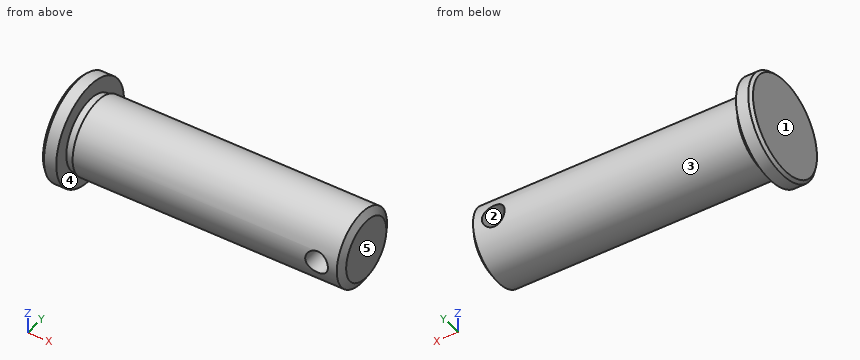
from build123d import *

# Parameters (mm, degrees)
CHAMFER_1_SIZE           = 1.5
CHAMFER_2_SIZE           = 4
CHAMFER_2_SIZE2          = 2.309401077
CUT_EXTRUDE_1_DEPTH      = 159.663165227
CUT_EXTRUDE_1_DEPTH_BACK = 159.663165227
SKETCH_2_R               = 6


with BuildPart() as part:
    # 草图1 → 旋转1 (revolve)
    with BuildSketch(Plane.XY, mode=Mode.PRIVATE) as revolve_1_sk:
        Polygon((0, 0), (154, 0), (154, 20), (12, 20), (12, 19), (8, 19), (8, 27), (0, 27), align=None)
    revolve(revolve_1_sk.sketch.rotate(Axis((-105.652173913, 0, 0), (1, 0, 0)), 90), axis=Axis((-105.652173913, 0, 0), (1, 0, 0)))

    # 倒角1
    chamfer_1_edges = [part.edges().sort_by_distance(p)[0] for p in [
        (0, 0, -27),
    ]]
    chamfer(chamfer_1_edges, length=CHAMFER_1_SIZE)

    # 倒角2
    chamfer_2_edges = [part.edges().sort_by_distance(p)[0] for p in [
        (154, 0, -20),
    ]]
    chamfer_2_side = [part.faces().sort_by_distance(p)[0] for p in [
        (154, 0, 0),
    ]]
    chamfer(chamfer_2_edges, length=CHAMFER_2_SIZE, length2=CHAMFER_2_SIZE2, reference=chamfer_2_side[0])

    # 草图2 → 切除-拉伸1 (cut, two sides: drawn at the far end of the back side and taken through both)
    with BuildSketch(Plane(origin=(0, 0, 0), x_dir=(1, 0, 0), z_dir=(0, 1, 0)).offset(-CUT_EXTRUDE_1_DEPTH_BACK)):
        with Locations(Location((141, 0, 0), (0, 0, 270))):
            Circle(SKETCH_2_R)
    extrude(amount=CUT_EXTRUDE_1_DEPTH + CUT_EXTRUDE_1_DEPTH_BACK, mode=Mode.SUBTRACT)


solid = part.part
Input: part model. Units: mm. Frame: model coordinates. Face numbers are marked on the shaded views. A direction names the side the tool comes from. Round coordinates to 2 decimals unless told otherwise and drop trailing zeros. Write each loop counter-clockwise with the first axis right and the second up, starting at its lowest first coordinate (ties: lowest second). Pieces come first, ordered by that corner, then holes.
1) Draft query along Z for the marked faces 1, 2 and 3. Return one class per face: pulls with the +Z half, pulls with the -Z half, needs draft (parallel to the pull), parting line crosses it, or undercut.
2) Reachability of the marked faces 4 and 5 from +Z, -Z, +X, -X, +Y, -Y: full face, straight path, thin tool, end or side. Return the list, or none.
3) Cut plane D-D (x = 141). Return the cut outline in (y, z).
4) Cut plane C-C (x = 36.5). Return the cut outline in (y, z), then the cut area to 3 significant figures.
5) Cut plane B-B (y = 0). Return the cut outline in (x, z), then the cut area to 3 significant figures.
6) Ray query, L1, parallel to X at y = -4, z = 0; L2, parallel to X at y = 6, z = -22; L3, parallel to Z at x = 141, y = -8. Return the intervals inside material, ascending.
7) Cut plane A-A (z = 0). Return the cut outline in (x, y).
8) Contact query for flat-ended pins moving along their axis: P1, Ø5, axis at x = 110, z = -4.5, coming from the -Y side; P2, Ø2, axis at x = 38.5, y = 2.5, coming from the -Z side; P3, Ø1.5, axis at x = 138, z = 7, coming from the +Y side. Output: stop coordinate, or through.
Geometry says:
1. face 1: needs draft
1. face 2: undercut
1. face 3: parting line crosses it
2. face 4: none
2. face 5: +Z, -Z, +X, +Y, -Y
3. outline: (-19.08, -6) arc R20 ccw to (19.08, -6) - close; (-19.08, 6) - (19.08, 6) arc R20 ccw to start
4. outline: circle Ø40 at (0, 0)
4. area: 1,260 mm2
5. outline: (0, -25.5) - (1.5, -27) - (8, -27) - (8, -19) - (12, -19) - (12, -20) - (151.69, -20) - (154, -16) - (154, 16) - (151.69, 20) - (12, 20) - (12, 19) - (8, 19) - (8, 27) - (1.5, 27) - (0, 25.5) - close; hole circle Ø12 at (141, 0)
5. area: 6,140 mm2
6. L1: x = 0 to 135, 147 to 154
6. L2: x = 0 to 8
6. L3: z = -18.33 to -6, 6 to 18.33
7. outline: (0, -25.5) - (1.5, -27) - (8, -27) - (8, -19) - (12, -19) - (12, -20) - (135, -20) - (135, 20) - (12, 20) - (12, 19) - (8, 19) - (8, 27) - (1.5, 27) - (0, 25.5) - close; (147, -20) - (151.69, -20) - (154, -16) - (154, 16) - (151.69, 20) - (147, 20) - close
8. P1: stops at y = -19.9
8. P2: stops at z = -19.94
8. P3: stops at y = 19
